For this review, take the finished solid that the model builds, in its own axes (mm). Face numbers are marked on the shaded views. Coordinates: 2 decimals unless noted, no trailing zeros. Loops run counter-clockwise (first coordinate to the right, second up) from the corner with the lowest first, then second, coordinate; pieces in that order, holes last. Notation, with made-up numbers: (46, 26) - (50, 26) arc R32 ccw to (50, 53) - close; hole circle Ø9 at (-6.75, -24.75). An arc over 180 degrees is marked (long way). Answer as a JSON object with one key per item and string values. Group by question number.
Item 1: Clearance check with flat-ended pins moving along their axes: pin 1 (6 mm diameter, centred on y = 8.5, z = -36, fed in from -X); pin 2 (4 mm diameter, centred on x = 46.5, z = 47, fed in from +Y); pin 3 (16 mm diameter, centred on x = 45.92, z = -110.87, fed in from -Y); pin 4 (5 mm diameter, centred on x = -50, y = -5, fed in from -Z). State where each tip first meets the part, or that it passes through.
Item 2: We need section C-C (y = 5.5). State how many separate pieces and enclosed holes the cut face has, then the cut area to 3 significant figures.
Item 3: We need section A-A (z = 0). Give the boundary of the cut face in (x, y).
Item 4: Mouldability with a two-part tool opening along Z and no side actions: class the marked faces 1 and 2 as released by +Z, released by -Z, zero draft, split by the parting line, or undercut.
Item 5: We need section B-B (x = 0). Give the boundary of the cut face in (y, z).
Item 6: To check wall thickness, follow line 1 (X direction, y = -3.5, z = -1); line 2 (X direction, y = 5.5, z = 40); line 3 (Z direction, x = -47, y = 4). State the ranges of each line that lie inside material, in increasing order.
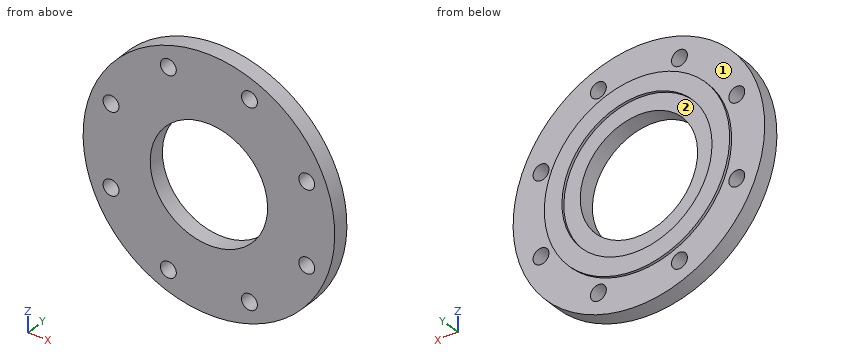
from build123d import *

# Parameters (mm, degrees)
SKETCH1_R           = 142.5
SKETCH1_R_2         = 66.5
BOSS_EXTRUDE1_DEPTH = 9.5
SKETCH2_R           = 105
SKETCH2_R_2         = 85
BOSS_EXTRUDE2_DEPTH = 3
SKETCH3_R           = 9
CUT_EXTRUDE1_DEPTH  = 203.41911965
CIRPATTERN1_COUNT   = 8


with BuildPart() as part:
    # Sketch1 → Boss-Extrude1 (new, symmetric)
    with BuildSketch(Plane(origin=(0, 0, 0), x_dir=(1, 0, 0), z_dir=(0, 1, 0))):
        with Locations(Location((0, 0, 0), (0, 0, 270))):
            Circle(SKETCH1_R)
        with Locations(Location((0, 0, 0), (0, 0, 270))):
            Circle(SKETCH1_R_2, mode=Mode.SUBTRACT)
    extrude(amount=BOSS_EXTRUDE1_DEPTH, both=True)

    # Sketch2 → Boss-Extrude2 (add)
    with BuildSketch(Plane(origin=(0, 9.5, 0), x_dir=(1, 0, 0), z_dir=(0, 1, 0))):
        with Locations(Location((0, 0, 0), (0, 0, 270))):
            Circle(SKETCH2_R)
        with Locations(Location((0, 0, 0), (0, 0, 270))):
            Circle(SKETCH2_R_2, mode=Mode.SUBTRACT)
    extrude(amount=BOSS_EXTRUDE2_DEPTH)

    # Sketch3 → Cut-Extrude1 (cut, through all)
    with BuildSketch(Plane(origin=(0, 9.5, 0), x_dir=(1, 0, 0), z_dir=(0, 1, 0))):
        with Locations(Location((-45.922011884, 110.865543901, 0), (0, 0, 270))):
            Circle(SKETCH3_R)
    cut_extrude1 = extrude(amount=-CUT_EXTRUDE1_DEPTH, mode=Mode.SUBTRACT)

    # CirPattern1: Cut-Extrude1 ×8 about axis
    cirpattern1_axis = Axis((0, 0, 0), (0, 1, 0))
    for i in range(1, CIRPATTERN1_COUNT):
        add(cut_extrude1.rotate(cirpattern1_axis, i * 360 / CIRPATTERN1_COUNT), mode=Mode.SUBTRACT)


solid = part.part
Check sheet entries:
{
 "1": {"pin 1": "stops at x = -138.63", "pin 2": "stops at y = 9.5", "pin 3": "passes through", "pin 4": "stops at z = -134.35"},
 "2": {"separate pieces": "1", "enclosed holes": "9", "area": "47,900 mm2"},
 "3": {"outline": "(-142.5, -9.5) - (-66.5, -9.5) - (-66.5, 9.5) - (-85, 9.5) - (-85, 12.5) - (-105, 12.5) - (-105, 9.5) - (-142.5, 9.5) - close; (66.5, -9.5) - (142.5, -9.5) - (142.5, 9.5) - (105, 9.5) - (105, 12.5) - (85, 12.5) - (85, 9.5) - (66.5, 9.5) - close"},
 "4": {"face 1": "zero draft", "face 2": "undercut"},
 "5": {"outline": "(-9.5, -142.5) - (9.5, -142.5) - (9.5, -105) - (12.5, -105) - (12.5, -85) - (9.5, -85) - (9.5, -66.5) - (-9.5, -66.5) - close; (-9.5, 66.5) - (9.5, 66.5) - (9.5, 85) - (12.5, 85) - (12.5, 105) - (9.5, 105) - (9.5, 142.5) - (-9.5, 142.5) - close"},
 "6": {"line 1": "x = -142.5 to -66.49, 66.49 to 142.5", "line 2": "x = -136.77 to -117.64, -104.09 to -53.12, 53.12 to 104.09, 117.64 to 136.77", "line 3": "z = -134.53 to -119.8, -101.93 to -47.05, 47.05 to 101.93, 119.8 to 134.53"}
}
